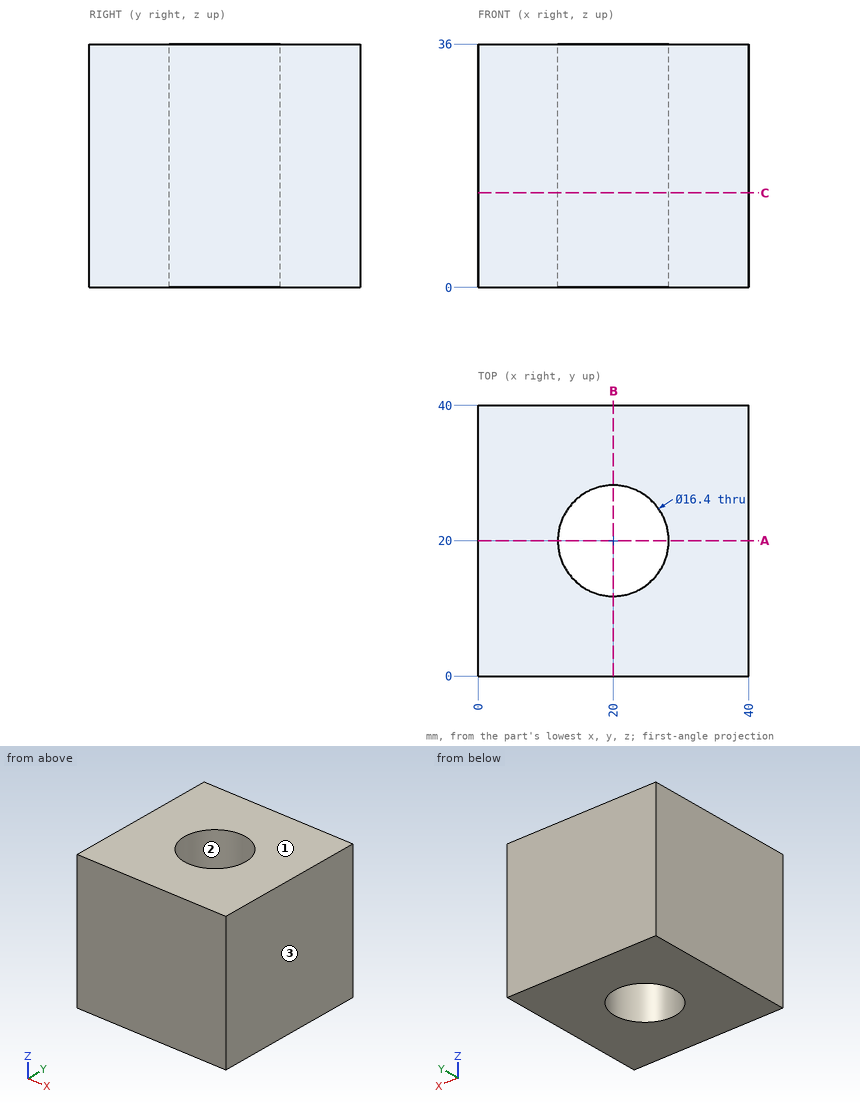
Answer from the drawing. Dimensions are ordinates in mm from the lowest x, y and z of the part. Round coordinates to 2 decimals unless told otherwise and drop trailing zeros. Order: outer loops, then holes, each group sorted by start corner. A loop starts at its lowest first (then second) coordinate and runs counter-clockwise, first axis right, second up.
1) A flat-ended cylindrical pin translates along its axis: pin 1 (13 mm diameter, centred on x = 20, y = 20, fed in from -Z). Find the tip coordinate at first contact, or state that the pin passes through.
2) Straight lines are drawn through the part: L1, parallel to Y at x = 20, z = 9; L2, parallel to X at y = 27.5, z = 14; L3, parallel to X at y = 14.5, z = 18.5. For each, find the intervals that lie inside material, in ascending order.
3) The part is cut by section A-A on y = 20. Write down the section's boundary in (x, z).
4) The part is cut by section C-C on z = 14. Write down the section's boundary in (x, y), plus the area to 3 significant figures.
5) The mould has two halves that part along X. Classify the marked faces 1, 2 and 3: released by +X, released by -X, zero draft, split by the parting line, or undercut.
Resolved:
1. pin 1: passes through
2. L1: y = 0 to 11.8, 28.2 to 40
2. L2: x = 0 to 16.68, 23.32 to 40
2. L3: x = 0 to 13.92, 26.08 to 40
3. outline: (0, 0) - (11.8, 0) - (11.8, 36) - (0, 36) - close; (28.2, 0) - (40, 0) - (40, 36) - (28.2, 36) - close
4. outline: (0, 0) - (40, 0) - (40, 40) - (0, 40) - close; hole circle Ø16.4 at (20, 20)
4. area: 1,390 mm2
5. face 1: zero draft
5. face 2: undercut
5. face 3: released by +X
